```python
from build123d import *

# Parameters (mm, degrees)
SKETCH1_W           = 40
SKETCH1_H           = 90
BOSS_EXTRUDE1_DEPTH = 6
SKETCH2_R           = 2.5
CUT_EXTRUDE1_DEPTH  = 6
SKETCH3_R           = 3
BOSS_EXTRUDE2_DEPTH = 6
BOSS_EXTRUDE3_START = 4
SKETCH4_R           = 3
BOSS_EXTRUDE3_DEPTH = 4


with BuildPart() as part:
    # Sketch1 → Boss-Extrude1 (new body)
    with BuildSketch(Plane.XY):
        Rectangle(SKETCH1_W, SKETCH1_H)
    extrude(amount=BOSS_EXTRUDE1_DEPTH)

    # Sketch2 → Cut-Extrude1 (cut)
    with BuildSketch(Plane.XY.offset(6)):
        with Locations((0, 38)):
            Circle(SKETCH2_R)
        with Locations((10, 38)):
            Circle(SKETCH2_R)
    extrude(amount=-CUT_EXTRUDE1_DEPTH, mode=Mode.SUBTRACT)

    # Sketch3 → Boss-Extrude2 (add)
    with BuildSketch(Plane.ZY.offset(20)):
        with BuildLine():
            Line((26, 45), (6, 45))
            Line((6, 45), (6, 33))
            Line((6, 33), (26, 33))
            ThreePointArc((26, 33), (32, 39), (26, 45))
        make_face()
        with Locations(Location((26, 39, 0), (0, 0, 270))):
            Circle(SKETCH3_R, mode=Mode.SUBTRACT)
    extrude(amount=-BOSS_EXTRUDE2_DEPTH)

    # Sketch4 → Boss-Extrude3 (add)
    with BuildSketch(Plane(origin=(0, 0, 0), x_dir=(0, 0, -1), z_dir=(1, 0, 0)).offset(BOSS_EXTRUDE3_START)):
        with BuildLine():
            Line((-21, -22.5), (-6, -22.5))
            Line((-6, -22.5), (-6, -37.5))
            Line((-6, -37.5), (-21, -37.5))
            ThreePointArc((-21, -37.5), (-28.5, -30), (-21, -22.5))
        make_face()
        with Locations((-21, -30)):
            Circle(SKETCH4_R, mode=Mode.SUBTRACT)
    boss_extrude3 = extrude(amount=BOSS_EXTRUDE3_DEPTH)

    # Mirror1: Boss-Extrude3 across plane
    add(boss_extrude3.mirror(Plane(origin=(0, 0, 0), x_dir=(0, 0, 1), z_dir=(1, 0, 0))))


solid = part.part
```
The listing builds one solid part. Answer for the finished solid, in the listing's coordinates (mm). A direction names the side the tool comes from. Give positions to 0.01 mm unless a question says otherwise; leave off trailing zeros. Loops run counter-clockwise (first coordinate to the right, second up) from the corner with the lowest first, then second, coordinate; pieces in that order, holes last. Notation, with made-up numbers: (52, -0.5) - (74, -0.5) arc R17 cw to (74, 23.5) - close; hole circle Ø6 at (14, 63.5). An arc over 180 degrees is marked (long way). Answer as CSV lines item,"result". Start each with the question number.
Item 1: A cutting plane is placed at A-A on x = 0. Determine the outline of the cut face in (y, z).
Item 2: Find the intervals of material crossed by line 1 (Z direction, x = -16.6, y = 39); line 2 (X direction, y = -25, z = 7); line 3 (Y direction, x = -5.75, z = 21), in increasing order. Write a range as from..to.
Item 3: A cutting plane is placed at C-C on x = -5.5. Determine the outline of the cut face in (y, z), then the cut area to 3 significant figures.
Item 4: Each of these flat-tipped pins is pushed along its axis until it touches: pin 1 (7.5 mm diameter, centred on y = -33, z = 18, fed in from +X); pin 2 (6 mm diameter, centred on y = 38, z = 19, fed in from +X); pin 3 (4.5 mm diameter, centred on y = -28, z = 15, fed in from -X). Where does it stop, or does it pass through?
Item 5: A cutting plane is placed at B-B on y = -30. Determine the outline of the cut face in (x, z).
Item 6: For faces 1 (the face through (20, -1, 3)), 2 (the face through (-17, 33, 16)), 3 (the face through (-14, 39, 19)), 4 (the face through (-8, -30, 17)), 5 (the face through (4, -30, 17)), determine the directions among +Z, -Z, +X, -X, +Y, -Y from which every point of the face is accessible in a straight line to the end or side of a thin tool.
Item 7: A cutting plane is placed at D-D on z = 8.5. Determine the outline of the cut face in (x, y).
Item 8: The mould has two halves that part along Y. Classify faces 6 (the face through (8, -30, 17)), 7 (the face through (-17, 39, 32)), 8 (the face through (9.46, 35.56, 3.04)), 9 (the face through (-6, -37.5, 13)): +Y half, -Y half, draft (parallel to the pull), parting line (faces both ways), or undercut.
Found:
1,outline,"(-45, 0) - (35.5, 0) - (35.5, 6) - (-45, 6) - close; (40.5, 0) - (45, 0) - (45, 6) - (40.5, 6) - close"
2,line 1,"z = 0..23, 29..32"
2,line 2,"x = -8..-4, 4..8"
2,line 3,"y = -37.5..-33, -27..-22.5"
3,outline,"(-45, 0) - (45, 0) - (45, 6) - (-22.5, 6) - (-22.5, 21) arc R7.5 ccw to (-37.5, 21) - (-37.5, 6) - (-45, 6) - close; hole circle Ø6 at (-30, 21)"
3,area,"825 mm^2"
4,pin 1,"stops at x = 8"
4,pin 2,"stops at x = -14"
4,pin 3,"stops at x = -8"
5,outline,"(-20, 0) - (20, 0) - (20, 6) - (8, 6) - (8, 18) - (4, 18) - (4, 6) - (-4, 6) - (-4, 18) - (-8, 18) - (-8, 6) - (-20, 6) - close; (-8, 24) - (-4, 24) - (-4, 28.5) - (-8, 28.5) - close; (4, 24) - (8, 24) - (8, 28.5) - (4, 28.5) - close"
6,face 1,"+Z, -Z, +X, +Y, -Y"
6,face 2,"+Z, +X, -X, -Y"
6,face 3,"+Z, +X, +Y, -Y"
6,face 4,"+Z, -X, +Y, -Y"
6,face 5,"+Z, +Y, -Y"
7,outline,"(-20, 33) - (-14, 33) - (-14, 45) - (-20, 45) - close; (-8, -37.5) - (-4, -37.5) - (-4, -22.5) - (-8, -22.5) - close; (4, -37.5) - (8, -37.5) - (8, -22.5) - (4, -22.5) - close"
8,face 6,"draft"
8,face 7,"parting line"
8,face 8,"undercut"
8,face 9,"-Y half"
